Source: CAD feature listing. Evaluate the final solid. Frame: model axes, mm. A direction names the side the tool comes from. Give positions to 0.01 mm unless a question says otherwise; leave off trailing zeros. Write each loop counter-clockwise with the first axis right and the second up, starting at its lowest first coordinate (ties: lowest second). Pieces come first, ordered by that corner, then holes. Notation, with made-up numbers: (40.5, 79) - (78.5, 79) arc R10 cw to (78.5, 87) - close; hole circle Ø2 at (-1.5, 44). An arc over 180 degrees is marked (long way). Answer as a JSON object with one key per item and string values. Group by question number.
from build123d import *

# Parameters (mm, degrees)
SKETCH1_R               = 3
SKETCH1_R_2             = 4
BOSS_EXTRUDE1_DEPTH     = 8
CUT_EXTRUDE1_DEPTH      = 8
CUT_EXTRUDE1_DEPTH_BACK = 16
SKETCH2_W               = 30
SKETCH2_H               = 6
SCALE1_SCALE            = 0.5


with BuildPart() as part:
    # Sketch1 → Boss-Extrude1 (new body)
    with BuildSketch(Plane.XY):
        with BuildLine():
            ThreePointArc((-50.757929877, -0.048790598), (-26.200561377, 4.481254982), (-1.442861384, 1.219054549))
            ThreePointArc((-1.442861384, 1.219054549), (3.282989256, -7.479585329), (-5.415650622, -12.205435969))
            ThreePointArc((-5.415650622, -12.205435969), (-25.840753116, -9.514120612), (-46.100582129, -13.251408215))
            ThreePointArc((-46.100582129, -13.251408215), (-55.030564812, -8.978773281), (-50.757929877, -0.048790598))
        make_face()
        with Locations((-48.429256003, -6.650099407)):
            Circle(SKETCH1_R, mode=Mode.SUBTRACT)
        with Locations((-3.429256003, -5.49319071)):
            Circle(SKETCH1_R_2, mode=Mode.SUBTRACT)
    extrude(amount=BOSS_EXTRUDE1_DEPTH)

    # Sketch2 → Cut-Extrude1 (cut, two sides: drawn at the far end of the back side and taken through both)
    with BuildSketch(Plane(origin=(0, 0, 0), x_dir=(1, 0, 0), z_dir=(0, 1, 0)).offset(-CUT_EXTRUDE1_DEPTH_BACK)):
        with Locations((3.570743997, -4)):
            Rectangle(SKETCH2_W, SKETCH2_H)
    extrude(amount=CUT_EXTRUDE1_DEPTH + CUT_EXTRUDE1_DEPTH_BACK, mode=Mode.SUBTRACT)


with BuildPart() as part_1:
    # Scale1: scaled about (0, 0, 0)
    add(part.part.scale(SCALE1_SCALE))


solid = part_1.part
Q1. First-contact query: pin 1 Ø0.9 at (y, z) = (-2, 1.5) entering from +X; pin 2 Ø1 at (x, z) = (-24.5, 2) entering from +Y; pin 3 Ø2 at (x, y) = (-3.5, -3) entering from -Z. Flat tips, straight axial feed; report the tip coordinate or a pass-through.
Q2. Section B-B on x = -0.25. Return the cut outline in (y, z), then the cut area to 3 significant figures.
Q3. Ray query, probe 1 along Z at (x, y) = (0, -4.75); probe 2 along X at (y, z) = (-2.75, 0.8); probe 3 along X at (y, z) = (-2.25, 3). Return the intervals inside material, ascending. Write a range as [from, to].
Q4. Section A-A on y = -4. Return the cut outline in (x, z), then the cut area to 3 significant figures.
Q5. Section C-C on y = -1.25. Return the cut outline in (x, z), then the cut area to 3 significant figures.
Q6. Reachability of faces 1 (the cylindrical face through (-12.776, -4.754, 1.972)), 2 (the flat face through (-5.715, -2, 2)) from +Z, -Z, +X, -X, +Y, -Y: full face, straight path, thin tool, end or side. Return the list, or none.
Q7. Section D-D on x = -4.5. Return the cut outline in (y, z).
Q8. Draft query along Y for faces 3 (the cylindrical face through (0.193, -2.146, 3.746)), 4 (the cylindrical face through (1.66, -3.67, 0.25)), 5 (the cylindrical face through (-16.055, 2.055, 1.972)). Return one class per face: released by +Y, released by -Y, zero draft, split by the parting line, or undercut.
Taken from the geometry:
{
 "1": {"pin 1": "stops at x = -5.71", "pin 2": "stops at y = 0.43", "pin 3": "stops at z = 0"},
 "2": {"outline": "(-5.93, 0) - (-4.11, 0) - (-4.11, 0.5) - (-5.93, 0.5) - close; (-5.93, 3.5) - (-4.11, 3.5) - (-4.11, 4) - (-5.93, 4) - close; (-1.38, 0) - (0.43, 0) - (0.43, 0.5) - (-1.38, 0.5) - close; (-1.38, 3.5) - (0.43, 3.5) - (0.43, 4) - (-1.38, 4) - close", "area": "3.63 mm²"},
 "3": {"probe 1": "z = [0, 0.5], [3.5, 4]", "probe 2": "x = [-27.67, -25.6], [-22.83, -5.71]", "probe 3": "x = [-27.55, -25.26], [-23.17, -5.71]"},
 "4": {"outline": "(-27.65, 0) - (-25.55, 0) - (-25.55, 4) - (-27.65, 4) - close; (-22.88, 0) - (-3.27, 0) - (-3.27, 0.5) - (-5.71, 0.5) - (-5.71, 3.5) - (-3.27, 3.5) - (-3.27, 4) - (-22.88, 4) - close; (-0.16, 0) - (1.55, 0) - (1.55, 0.5) - (-0.16, 0.5) - close; (-0.16, 3.5) - (1.55, 3.5) - (1.55, 4) - (-0.16, 4) - close", "area": "81.2 mm²"},
 "5": {"outline": "(-27.03, 0) - (-3.04, 0) - (-3.04, 0.5) - (-5.71, 0.5) - (-5.71, 3.5) - (-3.04, 3.5) - (-3.04, 4) - (-27.03, 4) - close; (-0.39, 0) - (1.45, 0) - (1.45, 0.5) - (-0.39, 0.5) - close; (-0.39, 3.5) - (1.45, 3.5) - (1.45, 4) - (-0.39, 4) - close", "area": "89.8 mm²"},
 "6": {"face 1": "+Z, -Z, -Y", "face 2": "+X, +Y, -Y"},
 "7": {"outline": "(-5.63, 0) - (1.53, 0) - (1.53, 0.5) - (-5.63, 0.5) - close; (-5.63, 3.5) - (1.53, 3.5) - (1.53, 4) - (-5.63, 4) - close"},
 "8": {"face 3": "undercut", "face 4": "split by the parting line", "face 5": "released by +Y"}
}
